Could you check a few things on this model? Use its own coordinates, in mm. A direction names the side the tool comes from. Round coordinates to 2 decimals unless told otherwise and drop trailing zeros. Loops run counter-clockwise (first coordinate to the right, second up) from the corner with the lowest first, then second, coordinate; pieces in that order, holes last. Notation, with made-up numbers: (58.25, 87) -> (75.25, 87) arc R26 cw to (75.25, 111) -> close; hole circle Ø10 at (-2, 11). An arc over 180 degrees is marked (long way). Write each question's results on one line, items separated by ' | '. Start each with the question number.
1) Imagine slicing it at A-A, the plane x = 0. Give the number of separate pieces and of enclosed holes in the cut face, plus the area to 3 significant figures.
2) For P1, Ø8, axis at y = 1, z = 6.5, coming from the -X side; P2, Ø7.5, axis at y = 0, z = -25, coming from the +X side; P3, Ø0.8, axis at x = 0, y = -7.5, coming from the +Z side; P4, Ø2, axis at y = -6.5, z = -18.5, coming from the +X side, each with a flat end and sliding along its axis, tell me the tip position at first contact or that it passes through.
3) Imagine slicing it at D-D, the plane z = 21. List the corners of the cut face in (x, y) for me, plus the area to 3 significant figures.
4) Which directions (+Z, -Z, +X, -X, +Y, -Y) give clear straight access to the entire face, cutting with the end or side of a thin tool? Please do faces 1 (the flat face through (0, 8, -20)), 2 (the flat face through (-7, -0.1, -27.3)), 3 (the flat face through (7, -0.1, 27.3)).
5) Imagine slicing it at B-B, the plane z = -25. List the corners of the cut face in (x, y) for me, plus the area to 3 significant figures.
6) We'd pull the mould along Y, two halves only. Please class faces 4 (the cylindrical face through (-8.49, 0.37, -19.5)), 5 (the conical face through (5.8, 5.8, 29.8)), 6 (the cylindrical face through (-0.098, 0.631, 27.003)), 7 (the flat face through (0, 0, 30)): pulls with the +Y half, pulls with the -Y half, needs draft (parallel to the pull), parting line crosses it, or undercut.
7) If I drill on probe 1 along Z at (x, y) = (6.75, -1.5); probe 2 along X at (y, z) = (-3.75, -22.5); probe 3 along Y at (x, z) = (-3.75, -25), over which ranges is the centre line in solid material (lowest first)?
from build123d import *

# Parameters (mm, degrees)
SKETCH_1_R           = 8.5
EXTRUDE_1_DEPTH      = 30
SKETCH_4_OUTSIDE_W   = 31.928
SKETCH_4_OUTSIDE_H   = 31.928
SKETCH_4_OUTSIDE_W_2 = 14
SKETCH_4_OUTSIDE_H_2 = 14
CUT_EXTRUDE_1_DEPTH  = 10
HOLE_WIZARD_M5_1_D   = 4.2
CHAMFER_1_SIZE       = 0.5
SKETCH_7_W           = 0.4
SKETCH_7_H           = 1.1


with BuildPart() as part:
    # 草图1 → 凸台-拉伸1 (new, symmetric)
    with BuildSketch(Plane.XY):
        Circle(SKETCH_1_R)
    extrude(amount=EXTRUDE_1_DEPTH, both=True)

    # 草图4 outside → 切除-拉伸1 (cut)
    with BuildSketch(Plane.XY.offset(30)):
        Rectangle(SKETCH_4_OUTSIDE_W, SKETCH_4_OUTSIDE_H)
        Rectangle(SKETCH_4_OUTSIDE_W_2, SKETCH_4_OUTSIDE_H_2, mode=Mode.SUBTRACT)
    cut_extrude_1 = extrude(amount=-CUT_EXTRUDE_1_DEPTH, mode=Mode.SUBTRACT)

    # M5 螺纹孔1 (through all)
    with Locations(Plane(origin=(7, 0, 0), x_dir=(0, 0, -1), z_dir=(1, 0, 0))):
        with Locations((-25, 0)):
            hole_wizard_m5_1 = Hole(HOLE_WIZARD_M5_1_D / 2)

    # 镜向1: 切除-拉伸1, M5 螺纹孔1 across plane
    add(cut_extrude_1.mirror(Plane.XY), mode=Mode.SUBTRACT)
    add(hole_wizard_m5_1.mirror(Plane.XY), mode=Mode.SUBTRACT)

    # 倒角1
    chamfer_1_edges = [part.edges().sort_by_distance(p)[0] for p in [
        (6.01040764, 6.01040764, -30),
        (6.01040764, 6.01040764, 30),
        (-6.01040764, 6.01040764, 30),
        (-6.01040764, 6.01040764, -30),
        (-6.01040764, -6.01040764, -30),
        (6.01040764, -6.01040764, -30),
        (-6.01040764, -6.01040764, 30),
        (6.01040764, -6.01040764, 30),
    ]]
    chamfer(chamfer_1_edges, length=CHAMFER_1_SIZE)

    # 草图7 → 切除-旋转1 (revolve, cut)
    with BuildSketch(Plane(origin=(0, 0, 0), x_dir=(1, 0, 0), z_dir=(0, 1, 0)), mode=Mode.PRIVATE) as cut_revolve_1_sk:
        with Locations((8.3, 17.05)):
            Rectangle(SKETCH_7_W, SKETCH_7_H)
    cut_revolve_1 = revolve(cut_revolve_1_sk.sketch.rotate(Axis((0, 0, -14.7653446), (0, 0, 1)), 180), axis=Axis((0, 0, -14.7653446), (0, 0, 1)), mode=Mode.SUBTRACT)

    # 镜向2: 切除-旋转1 across plane
    add(cut_revolve_1.mirror(Plane.XY), mode=Mode.SUBTRACT)


solid = part.part
Checked values:
1) separate pieces: 1 | enclosed holes: 2 | area: 931 mm^2
2) P1: x = -8.5 | P2: x = 7 | P3: z = 20 | P4: x = 6.48
3) outline: (-7, -4.82) arc R8.5 ccw to (-4.82, -7) -> (4.82, -7) arc R8.5 ccw to (7, -4.82) -> (7, 4.82) arc R8.5 ccw to (4.82, 7) -> (-4.82, 7) arc R8.5 ccw to (-7, 4.82) -> close | area: 188 mm^2
4) face 1: -Z, +X, -X, +Y | face 2: -Z, -X, +Y, -Y | face 3: +Z, +X, +Y, -Y
5) outline: (-7, -4.82) arc R8.5 ccw to (-4.82, -7) -> (4.82, -7) arc R8.5 ccw to (7, -4.82) -> (7, -2.1) -> (-7, -2.1) -> close; (-7, 2.1) -> (7, 2.1) -> (7, 4.82) arc R8.5 ccw to (4.82, 7) -> (-4.82, 7) arc R8.5 ccw to (-7, 4.82) -> close | area: 129 mm^2
6) face 4: parting line crosses it | face 5: pulls with the +Y half | face 6: undercut | face 7: needs draft
7) probe 1: -30 to -26.47, -23.53 to 23.53, 26.47 to 30 | probe 2: -7 to 7 | probe 3: -7 to -2.1, 2.1 to 7
